```python
from build123d import *

# Parameters (mm, degrees)
BOSS_EXTRUDE1_DEPTH   = 100
SHELL1_T              = -4
FILLET1_R             = 8.2
FILLET2_R             = 4.2
M8_TAPPED_HOLE1_D     = 6.8
M8_TAPPED_HOLE1_DEPTH = 19.75
M8_TAPPED_HOLE1_TIP   = 2.042926105


with BuildPart() as part:
    # Sketch1 → Boss-Extrude1 (new body)
    with BuildSketch(Plane.XY):
        Polygon((0, 0), (0, 208.736831721), (915, 1874.433314365), (1000, 1874.433314365), (1000, 1820.433314365), align=None)
    extrude(amount=BOSS_EXTRUDE1_DEPTH)

    # Shell1
    shell1_openings = [part.faces().sort_by_distance(p)[0] for p in [
        (0, 104.36841586, 50),
        (1000, 1847.433314365, 50),
    ]]
    offset(amount=SHELL1_T, openings=shell1_openings, kind=Kind.INTERSECTION)

    # Fillet1
    fillet1_edges = [part.edges().sort_by_distance(p)[0] for p in [
        (457.5, 1041.585073043, 100),
        (957.5, 1874.433314365, 100),
        (957.5, 1874.433314365, 0),
        (457.5, 1041.585073043, 0),
        (500, 910.216657182, 0),
        (500, 910.216657182, 100),
    ]]
    fillet(fillet1_edges, radius=FILLET1_R)

    # Fillet2
    fillet2_edges = [part.edges().sort_by_distance(p)[0] for p in [
        (958.683247588, 1870.433314365, 96),
        (458.683247588, 1035.431049715, 96),
        (500, 918.524703838, 96),
        (500, 918.524703838, 4),
        (458.683247588, 1035.431049715, 4),
        (958.683247588, 1870.433314365, 4),
    ]]
    fillet(fillet2_edges, radius=FILLET2_R)

    # M8 Tapped Hole1
    with Locations(Plane.XY.offset(100)):
        with Locations((316, 708.43)):
            Hole(M8_TAPPED_HOLE1_D / 2, depth=M8_TAPPED_HOLE1_DEPTH)
            with Locations((0, 0, -(M8_TAPPED_HOLE1_DEPTH + M8_TAPPED_HOLE1_TIP / 2))):  # 118° drill point
                Cone(0, M8_TAPPED_HOLE1_D / 2, M8_TAPPED_HOLE1_TIP, mode=Mode.SUBTRACT)


solid = part.part
```
Design review of the part built by this model. Coordinates are the model's own, in mm. A direction names the side the tool comes from. Coordinates: 2 decimals unless noted, no trailing zeros. Write each loop counter-clockwise with the first axis right and the second up, starting at its lowest first coordinate (ties: lowest second). Pieces come first, ordered by that corner, then holes.
1) Add section A-A (z = 34.5). Write out the cut boundary in (x, y).
2) To check wall thickness, follow L1, parallel to Z at x = 239.5, y = 626; L2, parallel to Y at x = 667, z = 78.5; L3, parallel to Y at x = 47.5, z = 58. State the ranges of each line that lie inside material, in increasing order.
3) Machinability: for faces 1 (the flat face through (502, 946, 0)), 2 (the flat face through (452.26, 1023.74, 49.41)), which of the approach directions +Z, -Z, +X, -X, +Y, -Y give a long, thin tool a straight path to every point of the face, cutting with its end or side? Answer none if there is none.
4) Mouldability with a two-part tool opening along Z and no side actions: class faces 3 (the cylindrical face through (451.5, 1019.74, 5.2)), 4 (the flat face through (451.095, 1029.925, 49.415)), 5 (the flat face through (502, 946, 4)), 6 (the cylindrical face through (462.41, 1045.67, 97.53)) as +Z half, -Z half, draft (parallel to the pull), parting line (faces both ways), or undercut.
5) Insertion check: pin 1 (4 mm diameter, centred on y = 496, z = 54.5, fed in from -X); pin 2 (4 mm diameter, centred on x = 851, z = 60.5, fed in from -Y); pin 3 (8 mm diameter, centred on x = 766.5, z = 71.5, fed in from +Y). Each pin has a flat end and moves straight along its axis. Give the tip position at first contact, or say it passes through.
Check result:
1. outline: (0, 0) - (1000, 1820.43) - (1000, 1828.74) - (0, 8.31) - close; (0, 200.43) - (917.37, 1870.43) - (1000, 1870.43) - (1000, 1874.43) - (915, 1874.43) - (0, 208.74) - close
2. L1: z = 0 to 4, 96 to 100
2. L2: y = 1214.23 to 1222.54, 1414.66 to 1422.97
2. L3: y = 86.47 to 94.78, 286.9 to 295.21
3. face 1: -Z, +X, -X, +Y, -Y
3. face 2: none
4. face 3: undercut
4. face 4: draft
4. face 5: undercut
4. face 6: +Z half
5. pin 1: stops at x = 156.7
5. pin 2: stops at y = 1545.55
5. pin 3: stops at y = 1611.38
